Geometry check sheet. Reference: drawing and pictorial views, mm from the part's lowest x, y, z. A direction names the side the tool comes from. Coordinates: 2 decimals unless noted, no trailing zeros. Write each loop counter-clockwise with the first axis right and the second up, starting at its lowest first coordinate (ties: lowest second). Pieces come first, ordered by that corner, then holes. Notation, with made-up numbers: (18, -19) -> (27, -19) arc R20 cw to (27, 7) -> close; hole circle Ø9 at (-37.5, 89.5). An arc over 180 degrees is marked (long way). Use a Markdown table: item, result. Add a question column.
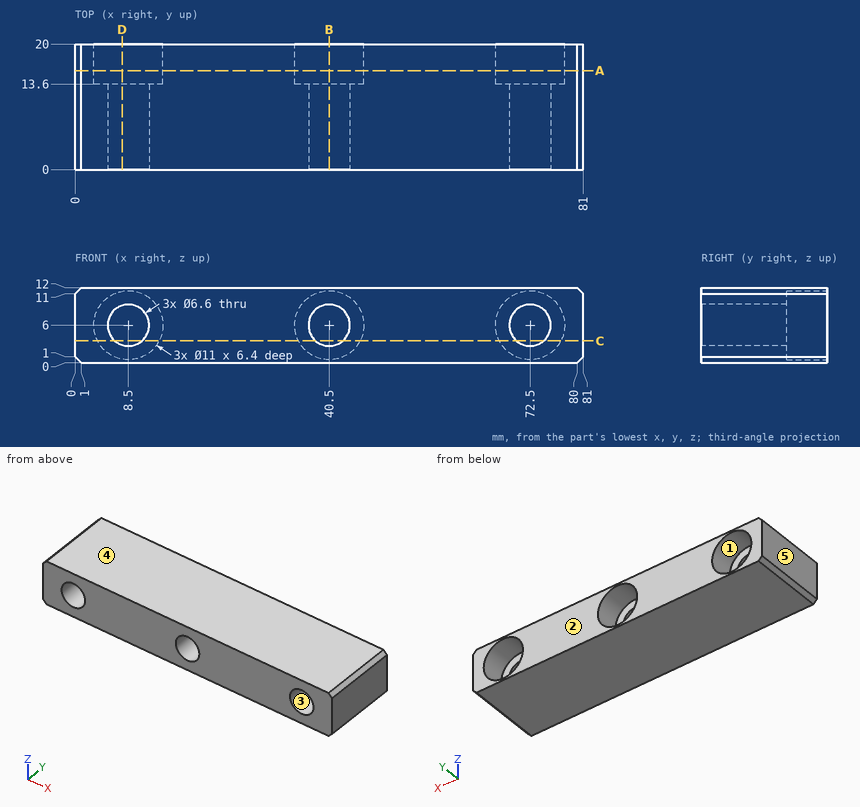
1) Thickness scan on L1, parallel to Z at x = 72.5, y = 10.75; L2, parallel to X at y = 14.25, z = 2; L3, parallel to X at y = 19.25, z = 9.25. Record the ranges inside material, lowest first.
2) Cross-section at B-B on x = 40.5. Record the boundary of the cut face in (y, z).
3) Cross-section at C-C on z = 3.5. Record the boundary of the cut face in (x, y), then the cut area to 3 significant figures.
4) Set-up check for the marked faces 1 and 2: record each of +Z, -Z, +X, -X, +Y, -Y from which the full face is reachable in a straight line by a thin tool's end or side.
5) Release check for a two-part mould opening along X. For the marked faces 3, 4 and 5 record: released by +X, released by -X, zero draft, split by the parting line, or undercut.
6) Gauge pin test, flat end, axial feed: pin 1 (6 mm diameter, centred on x = 72.5, z = 6, fed in from -Y). Record the tip position at first contact, or that the pin passes through.
7) Cross-section at A-A on y = 15.75. Record the boundary of the cut face in (x, z).
8) Cross-section at D-D on x = 7.5. Record the boundary of the cut face in (y, z), then the cut area to 3 significant figures.
Returned:
| question | item | result |
|---|---|---|
| 1 | L1 | z = 0 to 2.7, 9.3 to 12 |
| 1 | L2 | x = 0 to 4.73, 12.27 to 36.73, 44.27 to 68.73, 76.27 to 81 |
| 1 | L3 | x = 0 to 4.06, 12.94 to 36.06, 44.94 to 68.06, 76.94 to 81 |
| 2 | outline | (0, 0) -> (20, 0) -> (20, 0.5) -> (13.6, 0.5) -> (13.6, 2.7) -> (0, 2.7) -> close; (0, 9.3) -> (13.6, 9.3) -> (13.6, 11.5) -> (20, 11.5) -> (20, 12) -> (0, 12) -> close |
| 3 | outline | (0, 0) -> (6.35, 0) -> (6.35, 13.6) -> (3.6, 13.6) -> (3.6, 20) -> (0, 20) -> close; (10.65, 0) -> (38.35, 0) -> (38.35, 13.6) -> (35.6, 13.6) -> (35.6, 20) -> (13.4, 20) -> (13.4, 13.6) -> (10.65, 13.6) -> close; (42.65, 0) -> (70.35, 0) -> (70.35, 13.6) -> (67.6, 13.6) -> (67.6, 20) -> (45.4, 20) -> (45.4, 13.6) -> (42.65, 13.6) -> close; (74.65, 0) -> (81, 0) -> (81, 20) -> (77.4, 20) -> (77.4, 13.6) -> (74.65, 13.6) -> close |
| 3 | area | 1,260 mm² |
| 4 | face 1 | +Y |
| 4 | face 2 | +Z, -Z, +X, -X, +Y |
| 5 | face 3 | undercut |
| 5 | face 4 | zero draft |
| 5 | face 5 | released by -X |
| 6 | pin 1 | passes through |
| 7 | outline | (0, 1) -> (1, 0) -> (80, 0) -> (81, 1) -> (81, 11) -> (80, 12) -> (1, 12) -> (0, 11) -> close; hole circle Ø11 at (8.5, 6); hole circle Ø11 at (40.5, 6); hole circle Ø11 at (72.5, 6) |
| 8 | outline | (0, 0) -> (20, 0) -> (20, 0.59) -> (13.6, 0.59) -> (13.6, 2.86) -> (0, 2.86) -> close; (0, 9.14) -> (13.6, 9.14) -> (13.6, 11.41) -> (20, 11.41) -> (20, 12) -> (0, 12) -> close |
| 8 | area | 85.2 mm² |
